Part model, mm, in its own coordinate system. Face numbers are marked on the shaded views. A direction names the side the tool comes from. Round coordinates to 2 decimals unless told otherwise and drop trailing zeros. Write each loop counter-clockwise with the first axis right and the second up, starting at its lowest first coordinate (ties: lowest second). Pieces come first, ordered by that corner, then holes. Notation, with made-up numbers: (-17.5, 84.5) -> (12.5, 84.5) arc R14 cw to (12.5, 110.5) -> close; hole circle Ø10 at (73.25, 23.25). An arc over 180 degrees is marked (long way). Return JSON: item names as keys, results as strings. Group by question number.
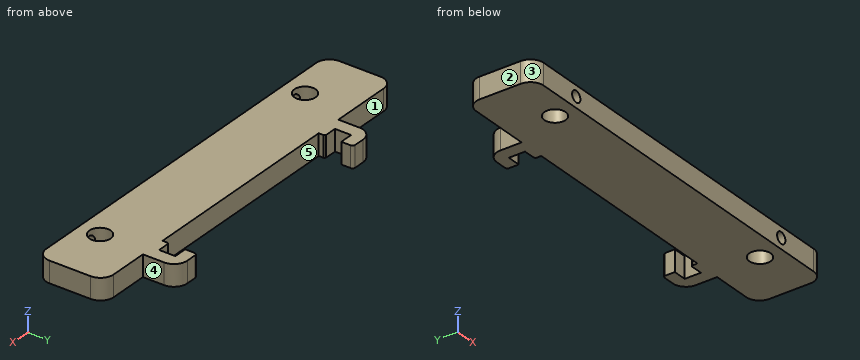
```python
from build123d import *

# Parameters (mm, degrees)
SKETCH1_W                      = 147
SKETCH1_H                      = 25.4
BOSS_EXTRUDE1_DEPTH            = 8
SKETCH2_W                      = 5
SKETCH2_H                      = 8
BOSS_EXTRUDE2_DEPTH            = 10
SKETCH3_W                      = 8
SKETCH3_H                      = 1.5
BOSS_EXTRUDE3_DEPTH            = 5
SKETCH4_W                      = 5
SKETCH4_H                      = 8
BOSS_EXTRUDE4_DEPTH            = 2.4
SKETCH7_R                      = 4
CUT_EXTRUDE1_DEPTH             = 150.392637034
SKETCH8_W                      = 10
SKETCH8_H                      = 8
BOSS_EXTRUDE5_DEPTH            = 3
FILLET1_R                      = 5
CHAMFER1_SIZE                  = 0.5
F_4_2_4_2_DIAMETER_HOLE1_D     = 4.2
F_4_2_4_2_DIAMETER_HOLE1_DEPTH = 9.5
F_4_2_4_2_DIAMETER_HOLE1_TIP   = 1.2618073
FILLET2_R                      = 5
FILLET3_R                      = 1


with BuildPart() as part:
    # Sketch1 → Boss-Extrude1 (new body)
    with BuildSketch(Plane.XY):
        with Locations((73.5, -12.7)):
            Rectangle(SKETCH1_W, SKETCH1_H)
    extrude(amount=BOSS_EXTRUDE1_DEPTH)

    # Sketch2 → Boss-Extrude2 (add)
    with BuildSketch(Plane(origin=(0, 0, 0), x_dir=(1, 0, 0), z_dir=(0, 1, 0))):
        with Locations((124.7, -4)):
            Rectangle(SKETCH2_W, SKETCH2_H)
        with Locations((30.5, -4)):
            Rectangle(SKETCH2_W, SKETCH2_H)
    extrude(amount=BOSS_EXTRUDE2_DEPTH)

    # Sketch3 → Boss-Extrude3 (add)
    with BuildSketch(Plane(origin=(33, 0, 0), x_dir=(0, 0, -1), z_dir=(1, 0, 0))):
        with Locations((-4, 9.25)):
            Rectangle(SKETCH3_W, SKETCH3_H)
    boss_extrude3 = extrude(amount=BOSS_EXTRUDE3_DEPTH)

    # Mirror1: Boss-Extrude3 across plane
    add(boss_extrude3.mirror(Plane(origin=(77.6, 0, 0), x_dir=(0, 0, 1), z_dir=(1, 0, 0))))

    # Sketch4 → Boss-Extrude4 (add)
    with BuildSketch(Plane(origin=(0, 0, 0), x_dir=(1, 0, 0), z_dir=(0, 1, 0))):
        with Locations((35.5, -4)):
            Rectangle(SKETCH4_W, SKETCH4_H)
        with Locations((119.7, -4)):
            Rectangle(SKETCH4_W, SKETCH4_H)
    extrude(amount=BOSS_EXTRUDE4_DEPTH)

    # Sketch7 → Cut-Extrude1 (cut, through all)
    with BuildSketch(Plane.XY.offset(8)):
        with Locations((21.5, -17.4)):
            Circle(SKETCH7_R)
        with Locations((125.5, -17.4)):
            Circle(SKETCH7_R)
    extrude(amount=-CUT_EXTRUDE1_DEPTH, mode=Mode.SUBTRACT)

    # Sketch8 → Boss-Extrude5 (add)
    with BuildSketch(Plane(origin=(0, 10, 0), x_dir=(1, 0, 0), z_dir=(0, 1, 0))):
        with Locations((33, -4)):
            Rectangle(SKETCH8_W, SKETCH8_H)
        with Locations((122.2, -4)):
            Rectangle(SKETCH8_W, SKETCH8_H)
    extrude(amount=BOSS_EXTRUDE5_DEPTH)

    # Fillet1
    fillet1_edges = [part.edges().sort_by_distance(p)[0] for p in [
        (28, 13, 4),
        (127.2, 13, 4),
        (0, 0, 4),
        (147, 0, 4),
    ]]
    fillet(fillet1_edges, radius=FILLET1_R)

    # Chamfer1
    chamfer1_edges = [part.edges().sort_by_distance(p)[0] for p in [
        (38, 2.4, 4),
        (117.2, 2.4, 4),
    ]]
    chamfer(chamfer1_edges, length=CHAMFER1_SIZE)

    # Ø4.2 (4.2) Diameter Hole1
    with Locations(Plane.XZ.offset(25.4)):
        with Locations((21.5, 4), (125.5, 4)):
            Hole(F_4_2_4_2_DIAMETER_HOLE1_D / 2, depth=F_4_2_4_2_DIAMETER_HOLE1_DEPTH)
            with Locations((0, 0, -(F_4_2_4_2_DIAMETER_HOLE1_DEPTH + F_4_2_4_2_DIAMETER_HOLE1_TIP / 2))):  # 118° drill point
                Cone(0, F_4_2_4_2_DIAMETER_HOLE1_D / 2, F_4_2_4_2_DIAMETER_HOLE1_TIP, mode=Mode.SUBTRACT)

    # Fillet2
    fillet2_edges = [part.edges().sort_by_distance(p)[0] for p in [
        (147, -25.4, 4),
        (0, -25.4, 4),
    ]]
    fillet(fillet2_edges, radius=FILLET2_R)

    # Fillet3
    fillet3_edges = [part.edges().sort_by_distance(p)[0] for p in [
        (38, 13, 4),
        (117.2, 13, 4),
    ]]
    fillet(fillet3_edges, radius=FILLET3_R)


solid = part.part
```
Item 1: Cut at C-C (x = 78.5). Write the cut outline in (y, z).
Item 2: Wall check: L1, parallel to X at y = -22.45, z = 4; L2, parallel to Y at x = 93, z = 2.75; L3, parallel to Y at x = 119.5, z = 6.5. Give the ranges that are in metal, low to high.
Item 3: Flat gauge pins, fed straight in: P1, Ø1, axis at y = 1, z = 3, coming from the -X side; P2, Ø2.5, axis at x = 64.5, z = 3.5, coming from the +Y side; P3, Ø4, axis at x = 21.5, z = 4, coming from the -Y side. Where does each tip first touch, or does it go through?
Item 4: Which spindle directions (+Z, -Z, +X, -X, +Y, -Y) get a long thin tool onto all of the face, cutting with end or side? Do the marked faces 1, 2, 3, 4 and 5. Say none if no direction does.
Item 5: Cut at A-A (x = 21.5). Write the cut outline in (y, z), then the cut area to 3 significant figures.
Item 6: Cut at B-B (y = -17.4). Write the cut outline in (x, z), then the cut area to 3 significant figures.
Checks:
{
 "1": {"outline": "(-25.4, 0) -> (0, 0) -> (0, 8) -> (-25.4, 8) -> close"},
 "2": {"L1": "x = 0.44 to 19.4, 23.6 to 123.4, 127.6 to 146.56", "L2": "y = -25.4 to 0", "L3": "y = -25.4 to 2.4, 8.5 to 13"},
 "3": {"P1": "stops at x = 28", "P2": "stops at y = 0", "P3": "stops at y = -13.94"},
 "4": {"face 1": "+Z, -Z, -X, +Y", "face 2": "+Z, -Z, -X, +Y, -Y", "face 3": "+Z, -Z, -X, -Y", "face 4": "+Z, -Z, +X, +Y", "face 5": "+Z, -Z, +Y"},
 "5": {"outline": "(-25.4, 0) -> (-21.4, 0) -> (-21.4, 1.9) -> (-25.4, 1.9) -> close; (-25.4, 6.1) -> (-21.4, 6.1) -> (-21.4, 8) -> (-25.4, 8) -> close; (-13.4, 0) -> (0, 0) -> (0, 8) -> (-13.4, 8) -> close", "area": "122 mm2"},
 "6": {"outline": "(0, 0) -> (17.5, 0) -> (17.5, 8) -> (0, 8) -> close; (25.5, 0) -> (121.5, 0) -> (121.5, 8) -> (25.5, 8) -> close; (129.5, 0) -> (147, 0) -> (147, 8) -> (129.5, 8) -> close", "area": "1,050 mm2"}
}
